Here's how the part is built. I have some questions about the finished solid (model axes, mm). A direction names the side the tool comes from. Round coordinates to 2 decimals unless told otherwise and drop trailing zeros. Write each loop counter-clockwise with the first axis right and the second up, starting at its lowest first coordinate (ties: lowest second). Pieces come first, ordered by that corner, then holes. Notation, with made-up numbers: (43.5, 16) - (89.5, 16) arc R26 cw to (89.5, 31) - close; hole circle Ø2 at (13.5, -16). An arc over 180 degrees is marked (long way). One line per item, written item: value. Start each with the question number.
Item 1: If I drill on line 1 (X direction, y = 150, z = -84.5); line 2 (Z direction, x = 78, y = 834) (3 decimals); line 3 (X direction, y = 2051, z = -7.5), over which ranges is the centre line in solid material (lowest first)?
Item 2: Imagine slicing it at A-A, the plane x = 36.5. Please give me the cut outline in (y, z) (3 decimals), then the cut area to 3 significant figures.
Item 3: For faces 5 (the face through (51, 1144, -92.175)), 6 (the face through (100, 1144, -48)), which set-ups out of +Z, -Z, +X, -X, +Y, -Y let a thin tool reach every point of the face, with its end or its side?
Item 4: Thinking about a two-plate mould opening in Z: for faces 1 (the face through (93.7, 1144, -48)), 2 (the face through (51, 1144, -98.475)), 3 (the face through (0, 1144, -49)), 4 (the face through (49, 1144, -4.775)), which applies, released by +Z, released by -Z, zero draft, split by the parting line, or undercut?
Item 5: Imagine slicing it at C-C, the plane y = 1573.5. Please give me the cut outline in (x, z) (3 decimals), then the cut area to 3 significant figures.
Item 6: Imagine slicing it at B-B, the plane z = -57.5. Please give me the cut outline in (x, y).
```python
from build123d import *

# Parameters (mm, degrees)
BOSS_EXTRUDE1_DEPTH = 2320


with BuildPart() as part:
    # Sketch2 → Boss-Extrude1 (new body)
    with BuildSketch(Plane(origin=(0, 0, 0), x_dir=(1, 0, 0), z_dir=(0, 1, 0))):
        with BuildLine():
            Line((7.875, -1.525), (92.125, -1.525))
            ThreePointArc((92.125, -1.525), (97.693465902, 0.781534098), (100, 6.35))
            Line((100, 6.35), (100, 90.6))
            ThreePointArc((100, 90.6), (97.693465902, 96.168465902), (92.125, 98.475))
            Line((92.125, 98.475), (7.875, 98.475))
            ThreePointArc((7.875, 98.475), (2.306534098, 96.168465902), (0, 90.6))
            Line((0, 90.6), (0, 6.35))
            ThreePointArc((0, 6.35), (2.306534098, 0.781534098), (7.875, -1.525))
        make_face()
        with BuildLine():
            Line((12.6, 4.775), (87.4, 4.775))
            ThreePointArc((87.4, 4.775), (91.854772721, 6.620227279), (93.7, 11.075))
            Line((93.7, 11.075), (93.7, 85.875))
            ThreePointArc((93.7, 85.875), (91.854772721, 90.329772721), (87.4, 92.175))
            Line((87.4, 92.175), (12.6, 92.175))
            ThreePointArc((12.6, 92.175), (8.145227279, 90.329772721), (6.3, 85.875))
            Line((6.3, 85.875), (6.3, 11.075))
            ThreePointArc((6.3, 11.075), (8.145227279, 6.620227279), (12.6, 4.775))
        make_face(mode=Mode.SUBTRACT)
    extrude(amount=BOSS_EXTRUDE1_DEPTH)


solid = part.part
```
Values follow:
1. line 1: x = 0 to 6.3, 93.7 to 100
1. line 2: z = -98.475 to -92.175, -4.775 to 1.525
1. line 3: x = 0 to 7.41, 92.59 to 100
2. outline: (0, -98.475) - (2320, -98.475) - (2320, -92.175) - (0, -92.175) - close; (0, -4.775) - (2320, -4.775) - (2320, 1.525) - (0, 1.525) - close
2. area: 29,200 mm^2
3. face 5: +Y, -Y
3. face 6: +Z, -Z, +X, +Y, -Y
4. face 1: undercut
4. face 2: released by -Z
4. face 3: zero draft
4. face 4: undercut
5. outline: (0, -90.6) arc R7.875 ccw to (7.875, -98.475) - (92.125, -98.475) arc R7.875 ccw to (100, -90.6) - (100, -6.35) arc R7.875 ccw to (92.125, 1.525) - (7.875, 1.525) arc R7.875 ccw to (0, -6.35) - close; hole (6.3, -85.875) arc R6.3 ccw to (12.6, -92.175) - (87.4, -92.175) arc R6.3 ccw to (93.7, -85.875) - (93.7, -11.075) arc R6.3 ccw to (87.4, -4.775) - (12.6, -4.775) arc R6.3 ccw to (6.3, -11.075) - close
5. area: 2,340 mm^2
6. outline: (0, 0) - (6.3, 0) - (6.3, 2320) - (0, 2320) - close; (93.7, 0) - (100, 0) - (100, 2320) - (93.7, 2320) - close
